Input: part model. Units: mm. Frame: model coordinates. A direction names the side the tool comes from. Coordinates: 2 decimals unless noted, no trailing zeros. Loops run counter-clockwise (first coordinate to the right, second up) from the corner with the lowest first, then second, coordinate; pieces in that order, holes last. Notation, with made-up numbers: (-10, 10.25) -> (18, 10.25) arc R22 ccw to (18, 37.25) -> close; hole circle Ø8 at (38.25, 20.25). An arc over 180 degrees is marked (long way). Put each result on its own line as item: value. Start each with the question number.
1) Cut plane D-D (y = -17). Return the cut outline in (x, z), plus the area to 3 significant figures.
2) Set-up query: faces 1 (the cylindrical face through (1.48, -26.4, -3.68)), 2 (the flat face through (2, 28, -22.25)), 3 (the flat face through (1, 4, -19.25)). Return all of +Z, -Z, +X, -X, +Y, -Y with unobstructed straight access to the full face (end or side cutting, diameter ignored); none if empty.
3) Material intervals for L1, parallel to Z at x = 1.7, y = -20.5; L2, parallel to Z at x = 0.35, y = -34; L3, parallel to Z at x = 2.15, y = 17.5, sorted ascending.
4) Cut plane C-C (x = 1.95). State how many separate pieces and enclosed holes the cut face has, plus the area to 3 significant figures.
5) Contact query for flat-ended pins moving along their axis: P1, Ø1, axis at x = 0.5, z = -8.5, coming from the -Y side; P2, Ø0.9, axis at x = 1.5, y = 2.5, coming from the -Z side; P3, Ø1.2, axis at x = 1.5, y = 27.5, coming from the +Z side. Output: stop coordinate, or through.
6) Cut plane B-B (z = -8). Return the cut outline in (x, y).
7) Pull-direction query (Z, two-part tool) for faces 4 (the cylindrical face through (1.521, 5.546, -13.649)), 5 (the cylindrical face through (1.48, -20.86, -15.71)), 6 (the flat face through (3, -10.4, -13.3)), 7 (the cylindrical face through (1.48, 16.8, -11.86)); classes: pulls with the +Z half, pulls with the -Z half, needs draft (parallel to the pull), parting line crosses it, or undercut.
8) Cut plane A-A (y = -29.75). Return the cut outline in (x, z), plus the area to 3 significant figures.
from build123d import *

# Parameters (mm, degrees)
SKETCH_1_R      = 1.55
SKETCH_1_R_2    = 1.3
EXTRUDE_1_DEPTH = 3
SKETCH_2_W      = 0.25
SKETCH_2_H      = 13.633784975
EXTRUDE_2_DEPTH = 3
FILLET_R2_1_R   = 2
FILLET_R1_2_R   = 1


with BuildPart() as part:
    # 草图1 → 凸台-拉伸1 (new body)
    with BuildSketch(Plane(origin=(0, 0, 0), x_dir=(0, 0, -1), z_dir=(1, 0, 0))):
        with BuildLine():
            Line((9.25, 19.75), (9.25, 6.116215025))
            Line((9.25, 6.116215025), (14.25, 6.116215025))
            Line((14.25, 6.116215025), (14.25, 0))
            ThreePointArc((14.25, 0), (3.04683438, -27.04683438), (-24, -38.25))
            Line((-24, -38.25), (-24, -39.7))
            Line((-24, -39.7), (5.238932767, -39.7))
            ThreePointArc((5.238932767, -39.7), (15.644467461, -21.049940647), (19.25, 0))
            Line((19.25, 0), (19.25, 19.75))
            Line((19.25, 19.75), (9.25, 19.75))
        make_face()
        with Locations((13, 15.75)):
            Circle(SKETCH_1_R, mode=Mode.SUBTRACT)
        with Locations((16.75, 5.25)):
            Circle(SKETCH_1_R, mode=Mode.SUBTRACT)
        with Locations((16.5, 11.05)):
            Circle(SKETCH_1_R_2, mode=Mode.SUBTRACT)
        with Locations((-1.828452918, -34.25)):
            Circle(SKETCH_1_R_2, mode=Mode.SUBTRACT)
        with Locations((8, -29.75)):
            Circle(SKETCH_1_R, mode=Mode.SUBTRACT)
        with Locations((10.756717193, -21.368448937)):
            Circle(SKETCH_1_R_2, mode=Mode.SUBTRACT)
        with Locations((14.615659071, -13.170834237)):
            Circle(SKETCH_1_R, mode=Mode.SUBTRACT)
        with Locations((16.57025586, -4.32369512)):
            Circle(SKETCH_1_R_2, mode=Mode.SUBTRACT)
    extrude(amount=EXTRUDE_1_DEPTH)

    # 草图2 → 凸台-拉伸2 (add, through all)
    with BuildSketch(Plane(origin=(3, 0, 0), x_dir=(0, 0, -1), z_dir=(1, 0, 0))):
        with Locations((9.125, 12.933107513)):
            Rectangle(SKETCH_2_W, SKETCH_2_H)
        with BuildLine():
            Line((12, 19.75), (19.25, 19.75))
            Line((19.25, 19.75), (19.25, 8.800075988))
            ThreePointArc((19.25, 8.800075988), (20.460820452, 15.653303833), (23.94667319, 21.676728835))
            ThreePointArc((23.94667319, 21.676728835), (24.913997325, 23.348229273), (25.25, 25.25))
            Line((25.25, 25.25), (25.25, 28.75))
            Line((25.25, 28.75), (22.25, 28.75))
            Line((22.25, 28.75), (22.25, 27.25))
            ThreePointArc((22.25, 27.25), (22.957106781, 25.542893219), (21.25, 26.25))
            Line((21.25, 26.25), (13.5, 26.25))
            Line((13.5, 26.25), (13.5, 23.75))
            ThreePointArc((13.5, 23.75), (14.366025404, 22.25), (12.633974596, 22.25))
            Line((12.633974596, 22.25), (12, 22.25))
            Line((12, 22.25), (12, 19.75))
        make_face()
    extrude(amount=-EXTRUDE_2_DEPTH)

    # R2 圆角1
    fillet_r2_1_edges = [part.edges().sort_by_distance(p)[0] for p in [
        (1.5, -39.7, -5.238932767),
        (1.5, 6.116215025, -14.25),
        (1.5, 19.75, -12),
    ]]
    fillet(fillet_r2_1_edges, radius=FILLET_R2_1_R)

    # R1 圆角2
    fillet_r1_2_edges = [part.edges().sort_by_distance(p)[0] for p in [
        (1.5, -38.25, 24),
        (1.5, 6.116215025, -9),
    ]]
    fillet(fillet_r1_2_edges, radius=FILLET_R1_2_R)


solid = part.part
Results found:
1. outline: (0, -16.92) -> (3, -16.92) -> (3, -10.26) -> (0, -10.26) -> close
1. area: 20.0 mm2
2. face 1: +Z, +X, -X
2. face 2: +Z, +X, -X, +Y
2. face 3: -Z, +X, -X, -Y
3. L1: z = -15.84 to -11.72, -9.79 to -8.29
3. L2: z = -9.33 to 0.55, 3.1 to 6.48
3. L3: z = -21.24 to -9
4. separate pieces: 1
4. enclosed holes: 8
4. area: 601 mm2
5. P1: stops at y = -36.01
5. P2: stops at z = -19.25
5. P3: stops at z = -22.25
6. outline: (0, -36.01) -> (3, -36.01) -> (3, -31.3) -> (0, -31.3) -> close; (0, -28.2) -> (3, -28.2) -> (3, -20.95) -> (0, -20.95) -> close
7. face 4: pulls with the +Z half
7. face 5: pulls with the -Z half
7. face 6: needs draft
7. face 7: undercut
8. outline: (0, -11.82) -> (3, -11.82) -> (3, -9.55) -> (0, -9.55) -> close; (0, -6.45) -> (3, -6.45) -> (3, -0.04) -> (0, -0.04) -> close
8. area: 26.0 mm2
